Source: three-view drawing plus pictorial views. Frame: mm from the lowest corner of the part. Coordinates: 2 decimals unless noted, no trailing zeros. Order: outer loops, then holes, each group sorted by start corner. A loop starts at its lowest first (then second) coordinate and runs counter-clockwise, first axis right, second up. Notation, with made-up numbers: (73.25, 79.5) - (81.25, 79.5) arc R19 ccw to (81.25, 88.5) - close; hole circle Ø2 at (88, 2.25). An arc over 180 degrees is marked (long way). One line per question, with ' | ' between items.
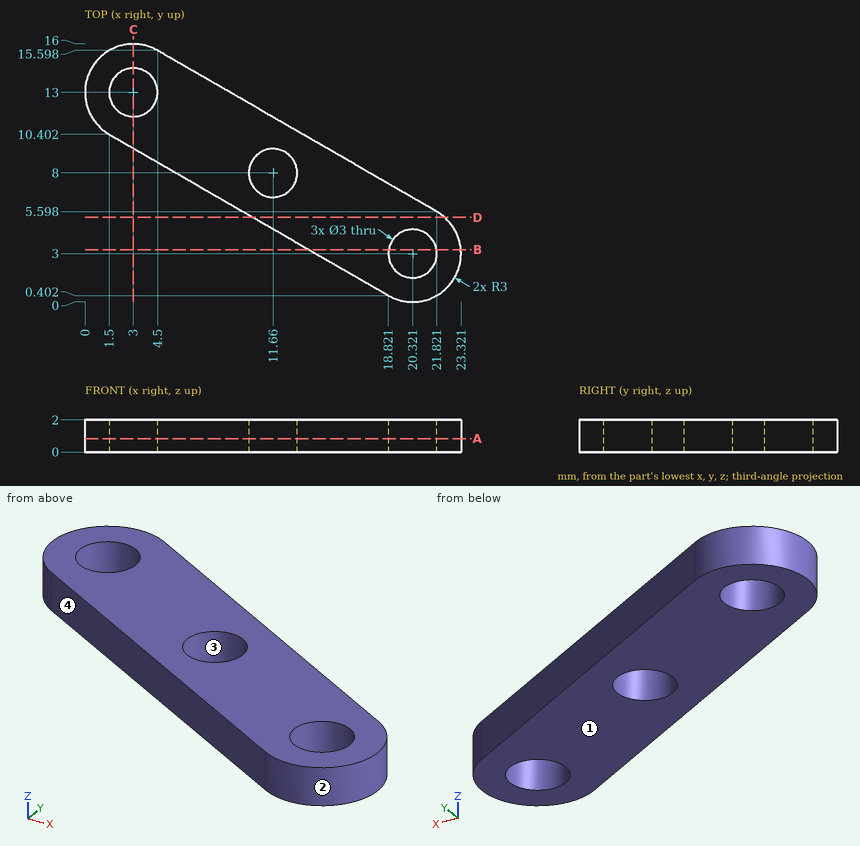
(1) Cut plane A-A (z = 0.85). Return the cut outline in (x, y).
Taken from the geometry:
outline: (1.5, 10.4) - (18.82, 0.4) arc R3 ccw to (21.82, 5.6) - (4.5, 15.6) arc R3 ccw to start; hole circle Ø3 at (3, 13); hole circle Ø3 at (11.66, 8); hole circle Ø3 at (20.32, 3)
(2) Pull-direction query (Y, two-part tool) for the marked faces 1, 2, 3 and 4; classes: pulls with the +Y half, pulls with the -Y half, needs draft (parallel to the pull), parting line crosses it, or undercut.
Taken from the geometry:
face 1: needs draft | face 2: parting line crosses it | face 3: undercut | face 4: pulls with the -Y half
(3) Pin query (flat end, axial travel): P1, Ø1.8, axis at x = 3, y = 13, coming from the +Z side; P2, Ø1, axis at x = 12, z = 1, coming from the -Y side. Return the tip coordinate at first contact, or that it passes through.
Taken from the geometry:
P1: passes through | P2: stops at y = 4.05
(4) Cut plane B-B (y = 3.25). Return the cut outline in (x, z), and give its area (3 significant figures).
Taken from the geometry:
outline: (13.89, 0) - (18.84, 0) - (18.84, 2) - (13.89, 2) - close; (21.8, 0) - (23.31, 0) - (23.31, 2) - (21.8, 2) - close | area: 12.9 mm²
(5) Cut plane D-D (y = 5.25). Return the cut outline in (x, z) (1 decimal).
Taken from the geometry:
outline: (10.4, 0) - (22.3, 0) - (22.3, 2) - (10.4, 2) - close
(6) Cut plane C-C (x = 3). Return the cut outline in (y, z) (1 decimal).
Taken from the geometry:
outline: (9.5, 0) - (11.5, 0) - (11.5, 2) - (9.5, 2) - close; (14.5, 0) - (16, 0) - (16, 2) - (14.5, 2) - close
(7) Material intervals for L1, parallel to X at y = 3.5, z = 0.65 (1 decimal); L2, parallel to Y at x = 3.25, z = 1.8; L3, parallel to X at y = 8, z = 0.9, sorted ascending. Write a range as from..to.
Taken from the geometry:
L1: x = 13.5..18.9, 21.7..23.3 | L2: y = 9.39..11.52, 14.48..15.99 | L3: x = 5.66..10.16, 13.16..17.66
